Could you check a few things on this drawing? It's one solid part, dimensions in mm from its lowest x, y, z. A direction names the side the tool comes from. Round coordinates to 2 decimals unless told otherwise and drop trailing zeros. Write each loop counter-clockwise with the first axis right and the second up, starting at its lowest first coordinate (ties: lowest second). Pieces come first, ordered by that corner, then holes. Notation, with made-up numbers: (18, 30) -> (75, 30) arc R30 cw to (75, 64) -> close; hole circle Ø7 at (-22.75, -7.75). An arc over 180 degrees is marked (long way). Answer in a Markdown table with one row per item.
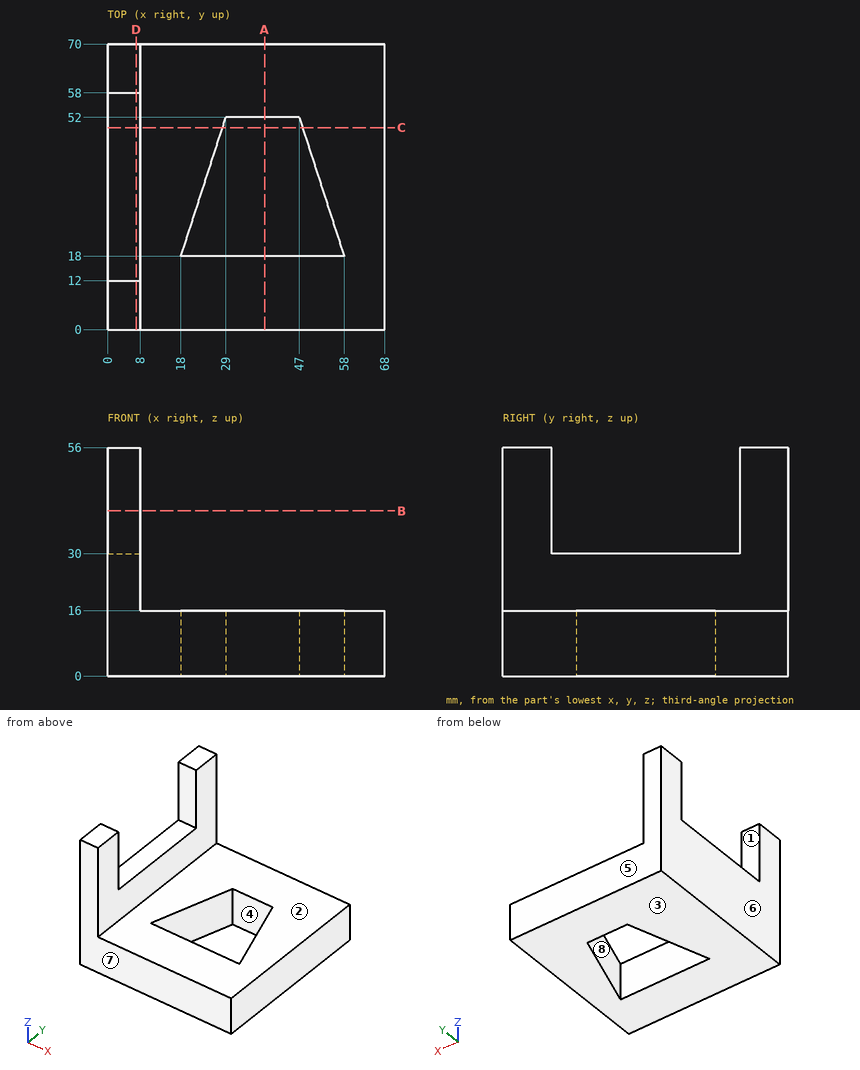
1) I want a section at A-A, the plane x = 38.5. List the corners of the cut face in (y, z) for me.
Response:
| item | result |
|---|---|
| outline | (0, 0) -> (18, 0) -> (18, 16) -> (0, 16) -> close; (52, 0) -> (70, 0) -> (70, 16) -> (52, 16) -> close |
2) We'd pull the mould along Y, two halves only. Please class the marked faces 5, 6, 7 and 8: +Y half, -Y half, draft (parallel to the pull), parting line (faces both ways), or undercut.
Response:
| item | result |
|---|---|
| face 5 | +Y half |
| face 6 | draft |
| face 7 | -Y half |
| face 8 | undercut |
3) I want a section at D-D, the plane x = 7. List the corners of the cut face in (y, z) for me, and give its area (3 significant figures).
Response:
| item | result |
|---|---|
| outline | (0, 0) -> (70, 0) -> (70, 56) -> (58, 56) -> (58, 30) -> (12, 30) -> (12, 56) -> (0, 56) -> close |
| area | 2,720 mm^2 |
4) I want a section at C-C, the plane y = 49.5. List the corners of the cut face in (x, z) for me, and give its area (3 significant figures).
Response:
| item | result |
|---|---|
| outline | (0, 0) -> (28.19, 0) -> (28.19, 16) -> (8, 16) -> (8, 30) -> (0, 30) -> close; (47.81, 0) -> (68, 0) -> (68, 16) -> (47.81, 16) -> close |
| area | 886 mm^2 |
5) For pin 1 (10 mm diameter, centred on y = 34, z = 37, fed in from -X); pin 2 (2.5 mm diameter, centred on x = 3.5, y = 32.5, fed in from +Z); pin 3 (18 mm diameter, centred on x = 40, y = 21.5, fed in from +Z), each with a flat end and sliding along its axis, tell me the tip position at first contact or that it passes through.
Response:
| item | result |
|---|---|
| pin 1 | passes through |
| pin 2 | stops at z = 30 |
| pin 3 | stops at z = 16 |
6) Which directions (+Z, -Z, +X, -X, +Y, -Y) give clear straight access to the entire face, cutting with the end or side of a thin tool? Please do the marked faces 1, 2, 3 and 4.
Response:
| item | result |
|---|---|
| face 1 | +Z, +X, -X |
| face 2 | +Z, +X, +Y, -Y |
| face 3 | -Z, +X, -X, +Y, -Y |
| face 4 | +Z, -Z |
7) I want a section at B-B, the plane z = 40.5. List the corners of the cut face in (x, y) for me, and give its area (3 significant figures).
Response:
| item | result |
|---|---|
| outline | (0, 0) -> (8, 0) -> (8, 12) -> (0, 12) -> close; (0, 58) -> (8, 58) -> (8, 70) -> (0, 70) -> close |
| area | 192 mm^2 |
8) I need wall thicknesses on line 1 (Y direction, x = 5, z = 31); line 2 (Z direction, x = 46, y = 61.5); line 3 (X direction, y = 43, z = 18). Which ranges of each line are inside material? Lowest first, please. Write a range as [from, to].
Response:
| item | result |
|---|---|
| line 1 | y = [0, 12], [58, 70] |
| line 2 | z = [0, 16] |
| line 3 | x = [0, 8] |
